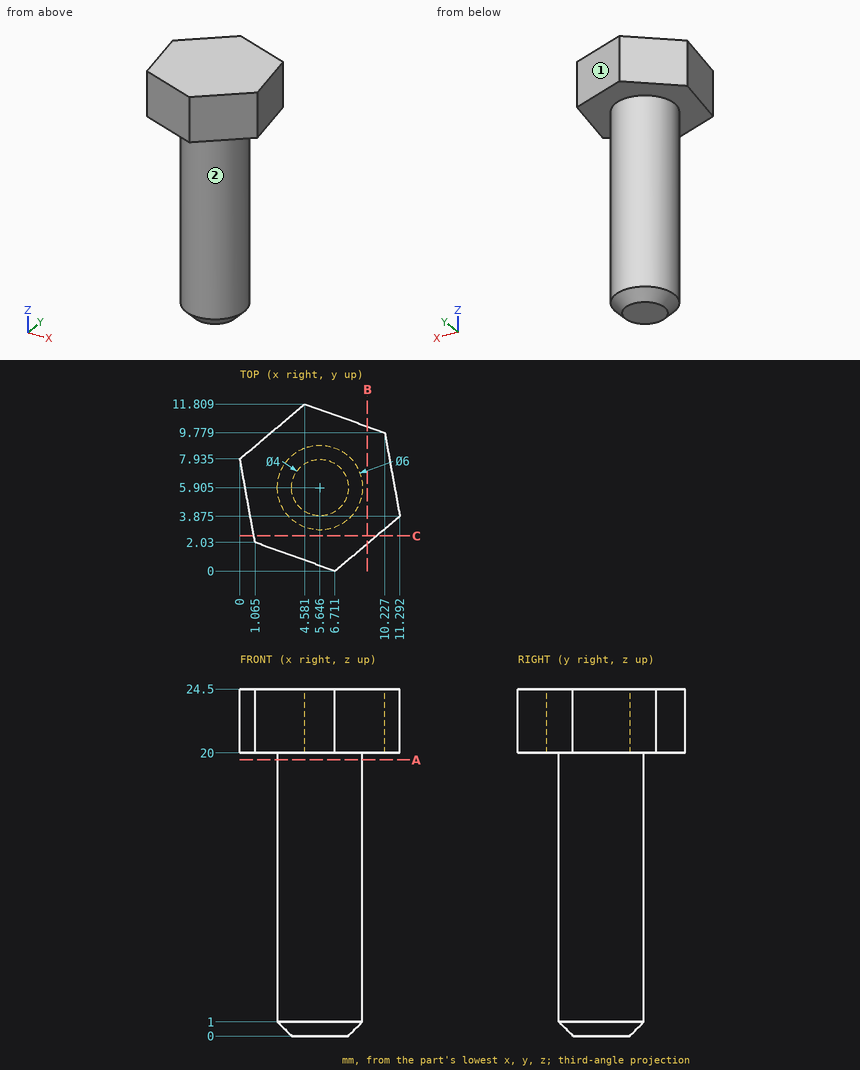
The drawing under review shows one solid part. Ordinate dimensions are in mm from its lowest x, y, z. A direction names the side the tool comes from. Give positions to 0.01 mm unless a question says otherwise; leave off trailing zeros. Order: outer loops, then holes, each group sorted by start corner. A loop starts at its lowest first (then second) coordinate and runs counter-clockwise, first axis right, second up. Notation, with made-up numbers: (-16, 6) - (-3, 6) arc R23 ccw to (-3, 36) - close; hole circle Ø4 at (65.5, 67). An arc over 180 degrees is marked (long way). Answer as a JSON object with one key per item and string values. Group by question number.
Item 1: Clearance check with flat-ended pins moving along their axes: pin 1 Ø4 at (y, z) = (2, 5.5) entering from -X; pin 2 Ø6 at (x, z) = (3, 9.5) entering from -Y (1 decimal); pin 3 Ø5 at (y, z) = (1.5, 10) entering from +X (1 decimal). State where each tip first meets the part, or that it passes through.
Item 2: Take a section at C-C on y = 2.5. Give the boundary of the cut face in (x, z).
Item 3: Take a section at A-A on z = 19.5. Give the boundary of the cut face in (x, y) (1 decimal).
Item 4: Wall thickness on line 1 along Z through (x, y) = (10, 8.75); line 2 along Y through (x, z) = (5.75, 5.5); line 3 along Y through (x, z) = (8, 7.75) (1 decimal): over which ranges is each line inside the solid? List them lowest first.
Item 5: Take a section at B-B on x = 9. Give the boundary of the cut face in (y, z) (1 decimal), and give its area (3 significant figures).
Item 6: Machinability: for the marked faces 1 and 2, which of the approach directions +Z, -Z, +X, -X, +Y, -Y give a long, thin tool a straight path to every point of the face, cutting with its end or side? Answer none if there is none.
Reported:
{
 "1": {"pin 1": "x = 3.33", "pin 2": "y = 2.9", "pin 3": "x = 8"},
 "2": {"outline": "(0.98, 20) - (9.67, 20) - (9.67, 24.5) - (0.98, 24.5) - close"},
 "3": {"outline": "circle Ø6 at (5.6, 5.9)"},
 "4": {"line 1": "20 to 24.5", "line 2": "2.91 to 8.9", "line 3": "4 to 7.8"},
 "5": {"outline": "(1.9, 20) - (10.2, 20) - (10.2, 24.5) - (1.9, 24.5) - close", "area": "37.3 mm^2"},
 "6": {"face 1": "+Z, -Z, +X, +Y", "face 2": "-Z"}
}
